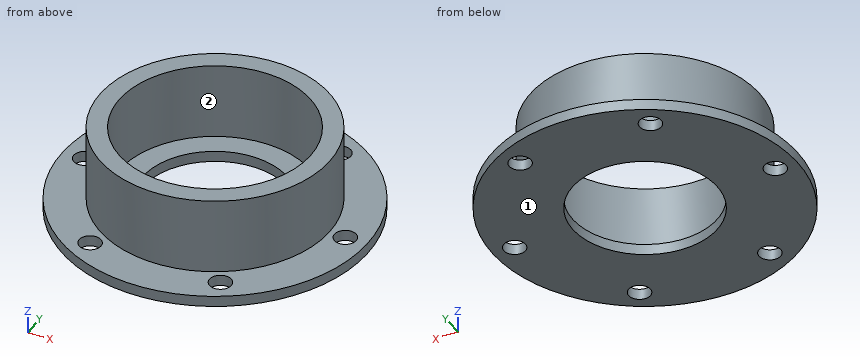
```python
from build123d import *

# Parameters (mm, degrees)
SKETCH_1_R          = 280
EXTRUDE_1_DEPTH     = 20
SKETCH_2_R          = 210
EXTRUDE_2_DEPTH     = 160
SKETCH_3_R          = 175
CUT_EXTRUDE_1_DEPTH = 140
SKETCH_4_R          = 20
CUT_EXTRUDE_3_DEPTH = 20
SKETCH_5_R          = 132.5
CUT_EXTRUDE_4_DEPTH = 20


with BuildPart() as part:
    # 草图1 → 凸台-拉伸1 (new body)
    with BuildSketch(Plane.XY):
        Circle(SKETCH_1_R)
    extrude(amount=EXTRUDE_1_DEPTH)

    # 草图2 → 凸台-拉伸2 (add)
    with BuildSketch(Plane.XY):
        Circle(SKETCH_2_R)
    extrude(amount=EXTRUDE_2_DEPTH)

    # 草图3 → 切除-拉伸1 (cut)
    with BuildSketch(Plane.XY.offset(160)):
        Circle(SKETCH_3_R)
    extrude(amount=-CUT_EXTRUDE_1_DEPTH, mode=Mode.SUBTRACT)

    # 草图4 → 切除-拉伸3 (cut)
    with BuildSketch(Plane.XY):
        with Locations((240, 0)):
            Circle(SKETCH_4_R)
        with Locations((-240, 0)):
            Circle(SKETCH_4_R)
        with Locations((-120, 207.846096908)):
            Circle(SKETCH_4_R)
        with Locations((120, 207.846096908)):
            Circle(SKETCH_4_R)
        with Locations((-120, -207.846096908)):
            Circle(SKETCH_4_R)
        with Locations((120, -207.846096908)):
            Circle(SKETCH_4_R)
    extrude(amount=CUT_EXTRUDE_3_DEPTH, mode=Mode.SUBTRACT)

    # 草图5 → 切除-拉伸4 (cut)
    with BuildSketch(Plane.XY):
        Circle(SKETCH_5_R)
    extrude(amount=CUT_EXTRUDE_4_DEPTH, mode=Mode.SUBTRACT)


solid = part.part
```
The model under review builds one solid part; all positions refer to its coordinate system, in mm. Face numbers are marked on the shaded views. A direction names the side the tool comes from. Coordinates: 2 decimals unless noted, no trailing zeros. Order: outer loops, then holes, each group sorted by start corner. A loop starts at its lowest first (then second) coordinate and runs counter-clockwise, first axis right, second up. Notation, with made-up numbers: M 37,5 L 62,5 A25 ccw 62,20 Z; hole C 34.5,57 d1. An arc over 180 degrees is marked long. One line per question, with ' | ' between items.
(1) Add section C-C, the plane y = -91.5. Write out the cut boundary in (x, z), then the cut area to 3 significant figures.
Geometry results:
outline: M -264.63,0 L -95.83,0 L -95.83,20 L -149.17,20 L -149.17,160 L -189.02,160 L -189.02,20 L -264.63,20 Z; M 95.83,0 L 264.63,0 L 264.63,20 L 189.02,20 L 189.02,160 L 149.17,160 L 149.17,20 L 95.83,20 Z | area: 17,900 mm²
(2) Add section A-A, the plane y = 0. Write out the cut boundary in (x, z), then the cut area to 3 significant figures.
Geometry results:
outline: M -280,0 L -260,0 L -260,20 L -280,20 Z; M -220,0 L -132.5,0 L -132.5,20 L -175,20 L -175,160 L -210,160 L -210,20 L -220,20 Z; M 132.5,0 L 220,0 L 220,20 L 210,20 L 210,160 L 175,160 L 175,20 L 132.5,20 Z; M 260,0 L 280,0 L 280,20 L 260,20 Z | area: 14,100 mm²
(3) Machinability: for the marked faces 1 and 2, which of the approach directions +Z, -Z, +X, -X, +Y, -Y give a long, thin tool a straight path to every point of the face, cutting with its end or side? Answer none if there is none.
Geometry results:
face 1: -Z, +X, -X, +Y, -Y | face 2: +Z
(4) Add section B-B, the plane x = -240. Write out the cut boundary in (y, z).
Geometry results:
outline: M -144.22,0 L -20,0 L -20,20 L -144.22,20 Z; M 20,0 L 144.22,0 L 144.22,20 L 20,20 Z
(5) Add section D-D, the plane x = 120. Write out the cut boundary in (y, z), then the cut area to 3 significant figures.
Geometry results:
outline: M -252.98,0 L -227.85,0 L -227.85,20 L -252.98,20 Z; M -187.85,0 L -56.18,0 L -56.18,20 L -127.38,20 L -127.38,160 L -172.34,160 L -172.34,20 L -187.85,20 Z; M 56.18,0 L 187.85,0 L 187.85,20 L 172.34,20 L 172.34,160 L 127.38,160 L 127.38,20 L 56.18,20 Z; M 227.85,0 L 252.98,0 L 252.98,20 L 227.85,20 Z | area: 18,900 mm²
(6) Insertion check: pin 1 (4 mm diameter, centred on y = -180, z = 117.5, fed in from -X); pin 2 (1.5 mm diameter, centred on x = -10, z = 73, fed in from -Y); pin 3 (2 mm diameter, centred on x = -140.5, y = 53, fed in from +Z). Each pin has a flat end and moves straight along its axis. Give the tip position at first contact, or say it passes through.
Geometry results:
pin 1: stops at x = -111.43 | pin 2: stops at y = -209.8 | pin 3: stops at z = 20
(7) For probe 1 along Y at (x, z) = (-120, 11.75); probe 2 along Y at (x, z) = (0, 89.5); probe 3 along Y at (x, z) = (0, 9.25), list the stretches that pass through material, from the lowest coordinate up. Write a range as from..to.
Geometry results:
probe 1: y = -252.98..-227.85, -187.85..-56.18, 56.18..187.85, 227.85..252.98 | probe 2: y = -210..-175, 175..210 | probe 3: y = -280..-132.5, 132.5..280
